Check sheet for the modelled part. Datum: model origin and axes. Units: mm. A direction names the side the tool comes from. Give positions to 0.01 mm unless a question says otherwise; leave off trailing zeros. Write each loop counter-clockwise with the first axis right and the second up, starting at its lowest first coordinate (ties: lowest second). Pieces come first, ordered by that corner, then holes. Notation, with made-up numbers: M 75.5,64 L 107.5,64 A33 ccw 107.5,101 Z; hole C -7,36 d1. An arc over 180 degrees is marked long. Write item = value, one per line. Start each with the question number.
1) Cross-section at B-B, the plane x = -44.45. Record the cut outline in (y, z), plus the area to 3 significant figures.
2) Access from +Z, -Z, +X, -X, +Y, -Y to the whole of each face (thin tool, end or side, straight path). Record for faces 1 (the flat face through (53, -52, 6)), 2 (the cylindrical face through (-32.9, -36.7, 8.1)).
3) Mould release check, pull along Y, two halves, no side actions. Record for faces 3 (the flat face through (-32, -35, 3)), 4 (the flat face through (-1, 55, 6)), 5 (the flat face through (-1, -55, 6)): released by +Y, released by -Y, zero draft, split by the parting line, or undercut.
4) Scan lines: line 1 along Y through (x, z) = (44.45, 10.25); line 2 along Y through (x, z) = (-32, 6.5); line 3 along X through (y, z) = (-32, 2.5). Record each from-to range of solid material in increasing order. Write a range as [from, to].
5) Go/stop test with flat-tipped pins: pin 1 (12 mm diameter, centred on x = 33, y = 30.5, fed in from -Z); pin 2 (5 mm diameter, centred on x = 33, y = 32.5, fed in from +Z). Record where each tip stops, or that it passes through.
6) Cross-section at A-A, the plane y = 0. Record the cut outline in (x, z).
```python
from build123d import *

# Parameters (mm, degrees)
SKETCH_1_W                   = 110
SKETCH_1_H                   = 110
EXTRUDE_1_DEPTH              = 13
SKETCH_2_R                   = 42.5
CUT_EXTRUDE_1_DEPTH          = 4
SKETCH_3_R                   = 26.5
CUT_EXTRUDE_2_DEPTH          = 79.860636569
EXTRUDE_START                = 3
SKETCH_4_R                   = 35
SKETCH_4_R_2                 = 26.5
EXTRUDE_2_DEPTH              = 3
HOLE_WIZARD_M8_1_D           = 6.8
CHAMFER_1_SIZE               = 5
HOLE_WIZARD_M5_1_D           = 5.8
HOLE_WIZARD_M5_1_CBORE_D     = 10
HOLE_WIZARD_M5_1_CBORE_DEPTH = 10
CHAMFER_2_SIZE               = 0.5


with BuildPart() as part:
    # 草图1 → 凸台-拉伸1 (new body)
    with BuildSketch(Plane.XY):
        Rectangle(SKETCH_1_W, SKETCH_1_H)
    extrude(amount=EXTRUDE_1_DEPTH)

    # 草图2 → 切除-拉伸1 (cut)
    with BuildSketch(Plane.XY.offset(13)):
        Circle(SKETCH_2_R)
    extrude(amount=-CUT_EXTRUDE_1_DEPTH, mode=Mode.SUBTRACT)

    # 草图3 → 切除-拉伸2 (cut, through all)
    with BuildSketch(Plane(origin=(0, 0, 0), x_dir=(-1, 0, 0), z_dir=(0, 0, -1))):
        Circle(SKETCH_3_R)
    extrude(amount=-CUT_EXTRUDE_2_DEPTH, mode=Mode.SUBTRACT)

    # 草图4 → 凸台-拉伸2 (add)
    with BuildSketch(Plane(origin=(0, 0, 0), x_dir=(-1, 0, 0), z_dir=(0, 0, -1)).offset(EXTRUDE_START)):
        with Locations(Location((0, 0, 0), (0, 0, 180))):
            Circle(SKETCH_4_R)
        Circle(SKETCH_4_R_2, mode=Mode.SUBTRACT)
    extrude(amount=-EXTRUDE_2_DEPTH)

    # M8 螺纹孔1 (through all)
    with Locations(Plane(origin=(0, 0, 0), x_dir=(-1, 0, 0), z_dir=(0, 0, -1))):
        with Locations((-44.45, 44.45), (44.45, 44.45), (44.45, -44.45), (-44.45, -44.45)):
            Hole(HOLE_WIZARD_M8_1_D / 2)

    # 倒角1
    chamfer_1_edges = [part.edges().sort_by_distance(p)[0] for p in [
        (55, -55, 6.5),
        (-55, -55, 6.5),
        (-55, 55, 6.5),
        (55, 55, 6.5),
    ]]
    chamfer(chamfer_1_edges, length=CHAMFER_1_SIZE)

    # M5 六角凹头螺钉的柱形沉头孔1 (through all)
    with Locations(Plane.XY.offset(13)):
        with Locations((-31.819805153, 31.819805153), (-31.819805153, -31.819805153), (31.819805153, -31.819805153), (31.819805153, 31.819805153)):
            CounterBoreHole(HOLE_WIZARD_M5_1_D / 2, HOLE_WIZARD_M5_1_CBORE_D / 2, HOLE_WIZARD_M5_1_CBORE_DEPTH)

    # 倒角2
    chamfer_2_edges = [part.edges().sort_by_distance(p)[0] for p in [
        (-35, 0, -3),
    ]]
    chamfer(chamfer_2_edges, length=CHAMFER_2_SIZE)


solid = part.part
```
Reply:
q1.outline = M -55,0 L -47.85,0 L -47.85,13 L -55,13 Z; M -41.05,0 L 41.05,0 L 41.05,13 L -41.05,13 Z; M 47.85,0 L 55,0 L 55,13 L 47.85,13 Z
q1.area = 1,250 mm2
q2.face_1 = +Z, -Z, +X, -Y
q2.face_2 = +Z
q3.face_3 = undercut
q3.face_4 = released by +Y
q3.face_5 = released by -Y
q4.line_1 = [-55, -47.85], [-41.05, 41.05], [47.85, 55]
q4.line_2 = [-55, -36.82], [-26.82, 26.82], [36.82, 55]
q4.line_3 = [-55, -34.71], [-28.93, 28.93], [34.71, 55]
q5.pin_1 = 0
q5.pin_2 = 3
q6.outline = M -55,0 L -35,0 L -35,-2.5 L -34.5,-3 L -26.5,-3 L -26.5,9 L -42.5,9 L -42.5,13 L -55,13 Z; M 26.5,-3 L 34.5,-3 L 35,-2.5 L 35,0 L 55,0 L 55,13 L 42.5,13 L 42.5,9 L 26.5,9 Z
